Model file for the job. Use its own axes, mm. Face numbers are marked on the shaded views. A direction names the side the tool comes from. Give positions to 0.01 mm unless a question says otherwise; leave off trailing zeros. Write each loop counter-clockwise with the first axis right and the second up, starting at its lowest first coordinate (ties: lowest second). Pieces come first, ordered by that corner, then holes. Notation, with made-up numbers: (75, 20) - (92, 20) arc R17 ccw to (92, 47) - close; hole circle Ø6 at (-37, 40.5). An arc over 180 degrees is marked (long way). One line per item, written item: value. Start each with the question number.
(1) Mould opens along X. For the marked faces 1, 2, 3 and 4 say: pulls with the +X half, pulls with the -X half, needs draft (parallel to the pull), parting line crosses it, or undercut.
(2) Cut at A-A, the plane z = 4.5. List the corners of the cut face in (x, y), and give its area (3 significant figures).
(3) Probe L1, parallel to Y at x = 0, z = 15; L2, parallel to Z at x = 6, y = 26; L3, parallel to X at y = -3.5, z = 29. List the from-to ranges inside material, lowest first.
(4) Cut at B-B, the plane x = 0. List the corners of the cut face in (y, z).
(5) Drop flat-ended pins along their axis: P1, Ø4, axis at x = -25, y = -1, coming from the -Z side; P2, Ø1.5, axis at x = 36.5, y = 35.5, coming from the -Z side. Give the stop position or say it passes through.
(6) 3-axis set-ups, long thin cutter, end or side, ignore diameter. For the marked faces 5 and 6: which of +Z, -Z, +X, -X, +Y, -Y reach the whole face in a straight line?
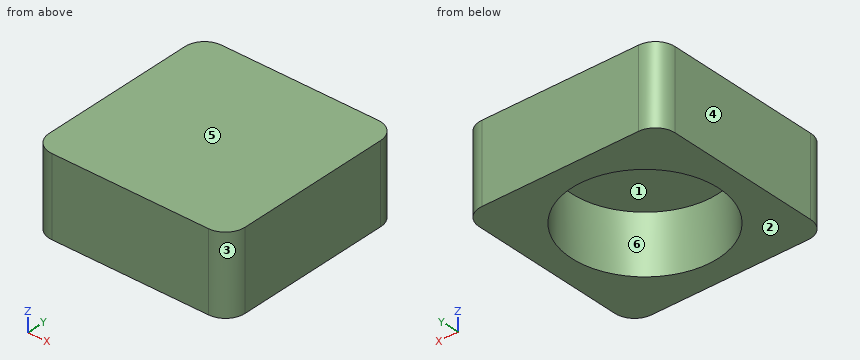
from build123d import *

# Parameters (mm, degrees)
SKETCH_1_W          = 100
SKETCH_1_H          = 100
EXTRUDE_1_DEPTH     = 40
SKETCH_2_R          = 37.5
CUT_EXTRUDE_1_DEPTH = 30
FILLET_1_R          = 10


with BuildPart() as part:
    # 草图1 → 凸台-拉伸1 (new body)
    with BuildSketch(Plane.XY):
        Rectangle(SKETCH_1_W, SKETCH_1_H)
    extrude(amount=EXTRUDE_1_DEPTH)

    # 草图2 → 切除-拉伸1 (cut)
    with BuildSketch(Plane(origin=(0, 0, 0), x_dir=(-1, 0, 0), z_dir=(0, 0, -1))):
        Circle(SKETCH_2_R)
    extrude(amount=-CUT_EXTRUDE_1_DEPTH, mode=Mode.SUBTRACT)

    # 圆角1
    fillet_1_edges = [part.edges().sort_by_distance(p)[0] for p in [
        (-50, -50, 20),
        (-50, 50, 20),
        (50, 50, 20),
        (50, -50, 20),
    ]]
    fillet(fillet_1_edges, radius=FILLET_1_R)


solid = part.part
Answers follow:
1. face 1: undercut
1. face 2: needs draft
1. face 3: pulls with the +X half
1. face 4: pulls with the -X half
2. outline: (-50, -40) arc R10 ccw to (-40, -50) - (40, -50) arc R10 ccw to (50, -40) - (50, 40) arc R10 ccw to (40, 50) - (-40, 50) arc R10 ccw to (-50, 40) - close; hole circle Ø75 at (0, 0)
2. area: 5,500 mm²
3. L1: y = -50 to -37.5, 37.5 to 50
3. L2: z = 30 to 40
3. L3: x = -50 to -37.34, 37.34 to 50
4. outline: (-50, 0) - (-37.5, 0) - (-37.5, 30) - (37.5, 30) - (37.5, 0) - (50, 0) - (50, 40) - (-50, 40) - close
5. P1: stops at z = 30
5. P2: stops at z = 0
6. face 5: +Z, +X, -X, +Y, -Y
6. face 6: -Z
